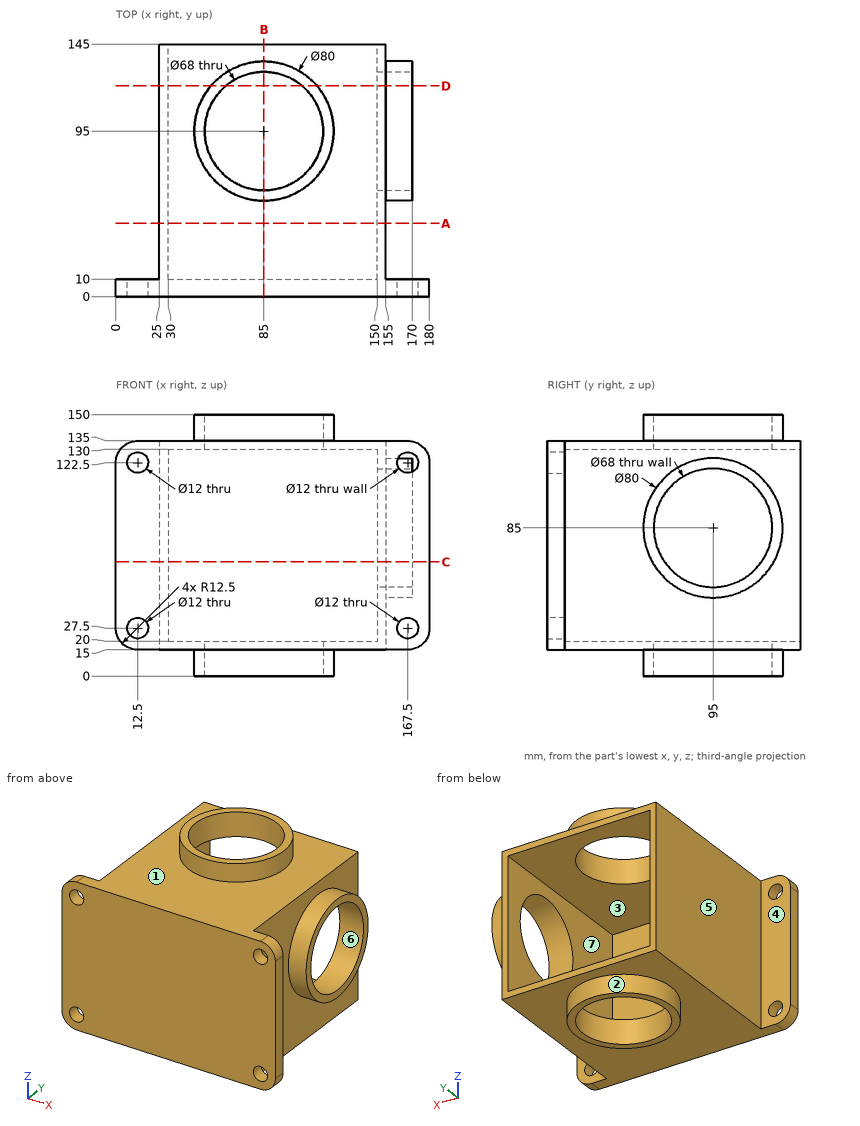
Here's the drawing with two shaded views (mm, measured from the low corner). I have some questions. A direction names the side the tool comes from. Round coordinates to 2 decimals unless told otherwise and drop trailing zeros. Loops run counter-clockwise (first coordinate to the right, second up) from the corner with the lowest first, then second, coordinate; pieces in that order, holes last. Notation, with made-up numbers: M 30.25,31.5 L 45.25,31.5 A11 cw 45.25,39.5 Z; hole C -14.75,26.5 d8. An arc over 180 degrees is marked long. Answer as CSV lines item,"result".
1) Imagine slicing it at B-B on x = 85. List the corners of the cut face in (y, z) for me.
From the geometry:
outline,"M 0,15 L 55,15 L 55,0 L 61,0 L 61,20 L 10,20 L 10,130 L 61,130 L 61,150 L 55,150 L 55,135 L 0,135 Z; M 129,0 L 135,0 L 135,15 L 145,15 L 145,20 L 129,20 Z; M 129,130 L 145,130 L 145,135 L 135,135 L 135,150 L 129,150 Z"
2) Imagine slicing it at A-A on y = 42. List the corners of the cut face in (x, z) for me, and give its area (3 significant figures).
From the geometry:
outline,"M 25,15 L 155,15 L 155,135 L 25,135 Z; hole M 30,20 L 150,20 L 150,130 L 30,130 Z"
area,"2,400 mm^2"
3) Imagine slicing it at D-D on y = 121. Count the separate pieces of the cut face and the enclosed holes in it, and give its area (3 significant figures).
From the geometry:
separate pieces,"3"
enclosed holes,"0"
area,"2,510 mm^2"
4) Which directions (+Z, -Z, +X, -X, +Y, -Y) give clear straight access to the entire face, cutting with the end or side of a thin tool? Please do the marked faces 1, 2, 3 and 4.
From the geometry:
face 1,"+Z"
face 2,"-Z"
face 3,"+Y"
face 4,"+Z, -Z, -X, +Y"
5) We'd pull the mould along X, two halves only. Please class the marked faces 5, 6 and 7: released by +X, released by -X, zero draft, split by the parting line, or undercut.
From the geometry:
face 5,"released by -X"
face 6,"zero draft"
face 7,"undercut"
6) For pin 1 Ø7 at (x, z) = (167.5, 27.5) entering from +Y; pin 2 Ø4 at (y, z) = (79, 97) entering from +X; pin 3 Ø12 at (y, z) = (75.5, 39) entering from +X; pin 4 Ø8 at (x, y) = (144.5, 45.5) entering from +Z, each with a flat end and sliding along its axis, tell me the tip position at first contact or that it passes through.
From the geometry:
pin 1,"through"
pin 2,"x = 30"
pin 3,"x = 155"
pin 4,"z = 135"
7) If I drill on probe 1 along X at (y, z) = (7.5, 122.5); probe 2 along Y at (x, z) = (165, 85); probe 3 along Z at (x, y) = (12, 5), over which ranges is the centre line in solid material (lowest first)?
From the geometry:
probe 1,"0 to 6.5, 18.5 to 161.5, 173.5 to 180"
probe 2,"0 to 10, 55 to 61, 129 to 135"
probe 3,"15.01 to 21.52, 33.48 to 116.52, 128.48 to 134.99"
8) Imagine slicing it at C-C on z = 65.5. List the corners of the cut face in (x, y) for me, and give its area (3 significant figures).
From the geometry:
outline,"M 0,0 L 180,0 L 180,10 L 155,10 L 155,60.08 L 170,60.08 L 170,67.15 L 150,67.15 L 150,10 L 30,10 L 30,145 L 25,145 L 25,10 L 0,10 Z; M 150,122.85 L 170,122.85 L 170,129.92 L 155,129.92 L 155,145 L 150,145 Z"
area,"3,080 mm^2"
